CAD build for the part. Positions are in the model's coordinates, mm. Face numbers are marked on the shaded views. A direction names the side the tool comes from. Round coordinates to 2 decimals unless told otherwise and drop trailing zeros. Loops run counter-clockwise (first coordinate to the right, second up) from the corner with the lowest first, then second, coordinate; pieces in that order, holes last.
from build123d import *

# Parameters (mm, degrees)
SKETCH1_R           = 14.5
BOSS_EXTRUDE1_DEPTH = 14
SKETCH2_R           = 11
BOSS_EXTRUDE2_DEPTH = 6
SKETCH3_R           = 20
BOSS_EXTRUDE3_DEPTH = 5
FILLET1_R           = 1
BOSS_EXTRUDE4_START = 12
SKETCH5_R           = 11
BOSS_EXTRUDE4_DEPTH = 12
SKETCH6_W           = 29
SKETCH6_H           = 36.6
BOSS_EXTRUDE5_DEPTH = 43


with BuildPart() as part:
    # Sketch1 → Boss-Extrude1 (new body)
    with BuildSketch(Plane(origin=(0, 0, 0), x_dir=(1, 0, 0), z_dir=(0, 1, 0))):
        with Locations(Location((0, 0, 0), (0, 0, 270))):
            Circle(SKETCH1_R)
    extrude(amount=BOSS_EXTRUDE1_DEPTH)

    # Sketch2 → Boss-Extrude2 (add)
    with BuildSketch(Plane(origin=(0, 14, 0), x_dir=(1, 0, 0), z_dir=(0, 1, 0))):
        with Locations(Location((0, 0, 0), (0, 0, 270))):
            Circle(SKETCH2_R)
    extrude(amount=BOSS_EXTRUDE2_DEPTH)

    # Sketch3 → Boss-Extrude3 (add)
    with BuildSketch(Plane(origin=(0, 20, 0), x_dir=(1, 0, 0), z_dir=(0, 1, 0))):
        with Locations(Location((0, 0, 0), (0, 0, 270))):
            Circle(SKETCH3_R)
    extrude(amount=BOSS_EXTRUDE3_DEPTH)

    # Sketch4 → Cut-Revolve1 (revolve, cut)
    with BuildSketch(Plane.XY, mode=Mode.PRIVATE) as cut_revolve1_sk:
        Polygon((-12, 25), (-20, 25), (-20, 23), align=None)
    revolve(cut_revolve1_sk.sketch.rotate(Axis((0, 0, 0), (0, 1, 0)), 270), axis=Axis((0, 0, 0), (0, 1, 0)), mode=Mode.SUBTRACT)

    # Fillet1
    fillet1_edges = [part.edges().sort_by_distance(p)[0] for p in [
        (-20, 23, 0),
        (0, 14, -14.5),
    ]]
    fillet(fillet1_edges, radius=FILLET1_R)

    # Sketch5 → Boss-Extrude4 (add)
    with BuildSketch(Plane.XZ.offset(BOSS_EXTRUDE4_START)):
        with Locations(Location((0, 0, 0), (0, 0, 90))):
            Circle(SKETCH5_R)
    extrude(amount=-BOSS_EXTRUDE4_DEPTH)

    # Sketch6 → Boss-Extrude5 (add)
    with BuildSketch(Plane.XZ.offset(12)):
        Rectangle(SKETCH6_W, SKETCH6_H)
    extrude(amount=BOSS_EXTRUDE5_DEPTH)


solid = part.part
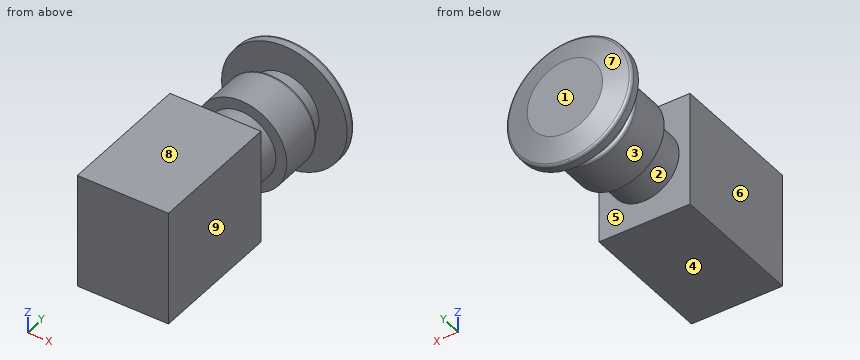
Item 1: Mould opens along Y. For the marked faces 1, 2, 3 and 4 say: released by +Y, released by -Y, zero draft, split by the parting line, or undercut.
Verdict:
face 1: released by +Y
face 2: undercut
face 3: undercut
face 4: zero draft
Item 2: 3-axis set-ups, long thin cutter, end or side, ignore diameter. For the marked faces 5, 6, 7, 8 and 9: which of +Z, -Z, +X, -X, +Y, -Y reach the whole face in a straight line?
Verdict:
face 5: none
face 6: +Z, -Z, -X, -Y
face 7: +Y
face 8: +Z, +X, -X, -Y
face 9: +Z, -Z, +X, -Y
Item 3: Wall check: L1, parallel to Y at x = -2, z = 11; L2, parallel to Y at x = -9, z = -11; L3, parallel to X at y = -49.5, z = 12.5. Give the ranges that are in metal, low to high.
Verdict:
L1: y = -55 to -12, 0 to 14, 20 to 25
L2: y = -55 to -12, 0 to 13.7, 20 to 24.45
L3: x = -14.5 to 14.5
Item 4: Flat gauge pins, fed straight in: P1, Ø8.5, axis at x = -7, y = -43.5, coming from the -Z side; P2, Ø12, axis at x = -2.5, y = -3, coming from the +Z side; P3, Ø8, axis at y = -13.5, z = -7.5, coming from the +X side; P4, Ø12, axis at x = 15, z = -9.5, coming from the +Y side. Where does each tip first touch, or does it go through?
Verdict:
P1: stops at z = -18.3
P2: stops at z = 14.5
P3: stops at x = 14.5
P4: stops at y = 25
Item 5: Cut at B-B (y = -41.5). List the corners of the cut face in (x, z).
Verdict:
outline: (-14.5, -18.3) - (14.5, -18.3) - (14.5, 18.3) - (-14.5, 18.3) - close
Item 6: Cut at A-A (y = -9). List the corners of the cut face in (x, z), plus the area to 3 significant figures.
Verdict:
outline: circle Ø22 at (0, 0)
area: 380 mm2
